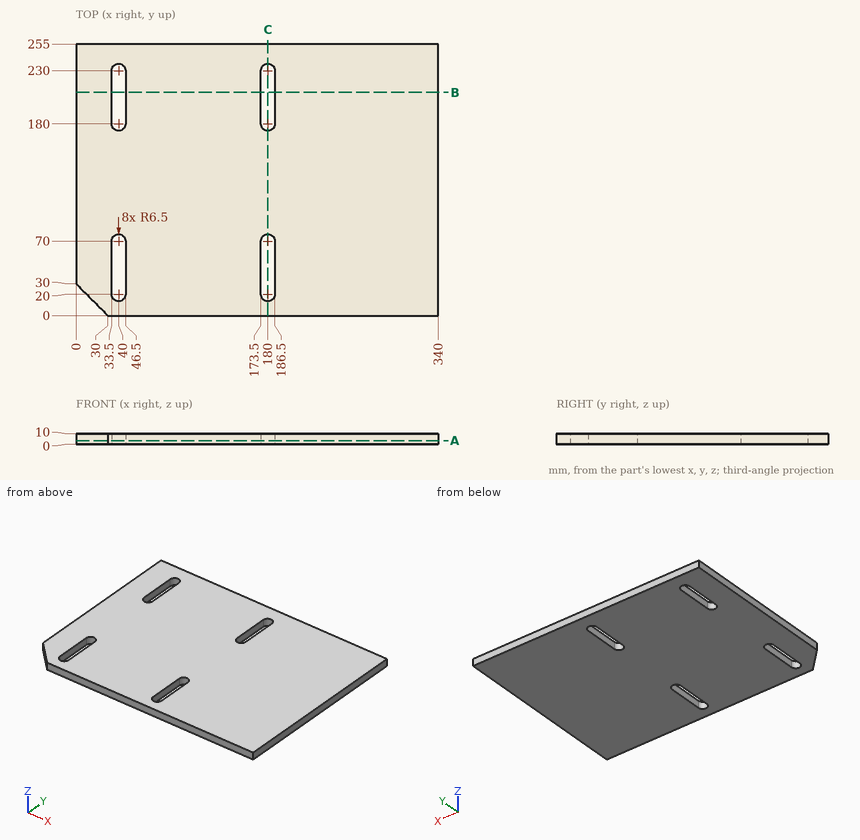
Geometry: see drawing. Coordinates: mm, zero at the bounding-box minimum. Round coordinates to 2 decimals unless told otherwise and drop trailing zeros. Write each loop counter-clockwise with the first axis right and the second up, starting at its lowest first coordinate (ties: lowest second). Pieces come first, ordered by that corner, then holes.
Item 1: Section query B-B (y = 209.5). Return loops of the section in (x, z), plus the area to 3 significant figures.
Item 2: Section query C-C (x = 180). Return loops of the section in (y, z), plus the area to 3 significant figures.
Item 3: Material intervals for L1, parallel to X at y = 53.5, z = 5.75; L2, parallel to Y at x = 43, z = 7; L3, parallel to X at y = 174.5, z = 8.25, sorted ascending.
Item 4: Pin query (flat end, axial travel): P1, Ø5, axis at y = 66, z = 3, coming from the -X side. Return the tip coordinate at first contact, or that it passes through.
Item 5: Section query A-A (z = 3.5). Return loops of the section in (x, y).
Completed:
1. outline: (0, 0) - (33.5, 0) - (33.5, 10) - (0, 10) - close; (46.5, 0) - (173.5, 0) - (173.5, 10) - (46.5, 10) - close; (186.5, 0) - (340, 0) - (340, 10) - (186.5, 10) - close
1. area: 3,140 mm2
2. outline: (0, 0) - (13.5, 0) - (13.5, 10) - (0, 10) - close; (76.5, 0) - (173.5, 0) - (173.5, 10) - (76.5, 10) - close; (236.5, 0) - (255, 0) - (255, 10) - (236.5, 10) - close
2. area: 1,290 mm2
3. L1: x = 0 to 33.5, 46.5 to 173.5, 186.5 to 340
3. L2: y = 0 to 14.23, 75.77 to 174.23, 235.77 to 255
3. L3: x = 0 to 36.54, 43.46 to 176.54, 183.46 to 340
4. P1: stops at x = 0
5. outline: (0, 30) - (30, 0) - (340, 0) - (340, 255) - (0, 255) - close; hole (33.5, 20) arc R6.5 ccw to (46.5, 20) - (46.5, 70) arc R6.5 ccw to (33.5, 70) - close; hole (33.5, 180) arc R6.5 ccw to (46.5, 180) - (46.5, 230) arc R6.5 ccw to (33.5, 230) - close; hole (173.5, 20) arc R6.5 ccw to (186.5, 20) - (186.5, 70) arc R6.5 ccw to (173.5, 70) - close; hole (173.5, 180) arc R6.5 ccw to (186.5, 180) - (186.5, 230) arc R6.5 ccw to (173.5, 230) - close
